Could you check a few things on this model? Use its own coordinates, in mm. Face numbers are marked on the shaded views. A direction names the side the tool comes from. Give positions to 0.01 mm unless a question says otherwise; leave off trailing zeros. Order: outer loops, then holes, each group sorted by start corner. A loop starts at its lowest first (then second) coordinate and runs counter-clockwise, first axis right, second up.
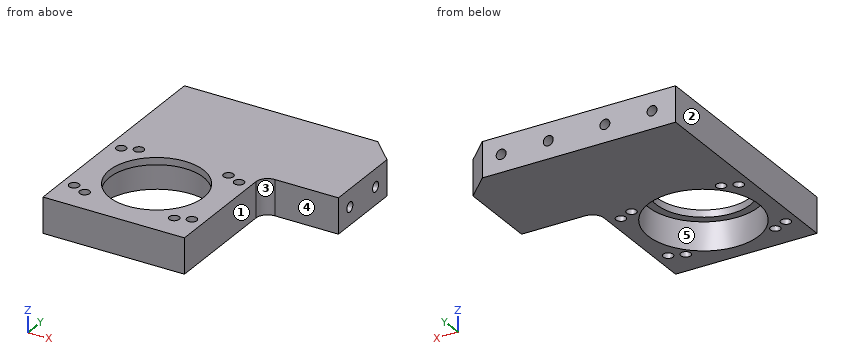
from build123d import *

# Parameters (mm, degrees)
SKETCH_1_W             = 110
SKETCH_1_H             = 100
EXTRUDE_1_DEPTH        = 7.5
SKETCH_10_R            = 23.5
CUT_EXTRUDE_1_DEPTH    = 12
SKETCH_12_R            = 20
CUT_EXTRUDE_2_DEPTH    = 76.292761936
SKETCH_13_W            = 50
SKETCH_13_H            = 55
CUT_EXTRUDE_3_DEPTH    = 76.828754441
FILLET_1_R             = 5
HOLE_WIZARD_M5_1_D     = 4.2
HOLE_WIZARD_M5_2_D     = 4.2
MOVE_FACE_1_BY         = 1
MOVE_FACE_2_BY         = 18
HOLE_WIZARD_M5_3_D     = 4.2
HOLE_WIZARD_M5_3_DEPTH = 12.4
HOLE_WIZARD_M5_3_TIP   = 1.2618073
HOLE_WIZARD_M5_4_D     = 4.2
HOLE_WIZARD_M5_4_DEPTH = 12.4
HOLE_WIZARD_M5_4_TIP   = 1.2618073
CHAMFER_2_SIZE         = 10


with BuildPart() as part:
    # 草图1 → 凸台-拉伸1 (new, symmetric)
    with BuildSketch(Plane.XY):
        Rectangle(SKETCH_1_W, SKETCH_1_H)
    extrude(amount=EXTRUDE_1_DEPTH, both=True)

    # 草图10 → 切除-拉伸1 (cut)
    with BuildSketch(Plane.XY.offset(-7.5)):
        with Locations((-25, -20)):
            Circle(SKETCH_10_R)
    extrude(amount=CUT_EXTRUDE_1_DEPTH, mode=Mode.SUBTRACT)

    # 草图12 → 切除-拉伸2 (cut, through all)
    with BuildSketch(Plane(origin=(0, 0, 4.5), x_dir=(-1, 0, 0), z_dir=(0, 0, -1))):
        with Locations((25, -20)):
            Circle(SKETCH_12_R)
    extrude(amount=-CUT_EXTRUDE_2_DEPTH, mode=Mode.SUBTRACT)

    # 草图13 → 切除-拉伸3 (cut, through all)
    with BuildSketch(Plane.XY.offset(7.5)):
        with Locations((30, -22.5)):
            Rectangle(SKETCH_13_W, SKETCH_13_H)
    extrude(amount=-CUT_EXTRUDE_3_DEPTH, mode=Mode.SUBTRACT)

    # 圆角1
    fillet_1_edges = [part.edges().sort_by_distance(p)[0] for p in [
        (5, 5, 0),
    ]]
    fillet(fillet_1_edges, radius=FILLET_1_R)

    # M5 螺纹孔1 (through all)
    with Locations(Plane(origin=(0, 0, -7.5), x_dir=(-1, 0, 0), z_dir=(0, 0, -1))):
        with Locations((0, -3.5), (0, -36.5), (50, -36.5), (50, -3.5)):
            Hole(HOLE_WIZARD_M5_1_D / 2)

    # M5 螺纹孔2 (through all)
    with Locations(Plane.XY.offset(7.5)):
        with Locations((-44, -1), (-44, -39), (-6, -39), (-6, -1)):
            Hole(HOLE_WIZARD_M5_2_D / 2)

    # Move Face 1: a face moved inward by 1.0
    extrude(part.faces().sort_by_distance((0, 50, 0))[0], amount=MOVE_FACE_1_BY, dir=(0, -1, 0), mode=Mode.SUBTRACT)

    # Move Face 2: a face moved inward by 18.0
    extrude(part.faces().sort_by_distance((55, 27, 0))[0], amount=MOVE_FACE_2_BY, dir=(-1, 0, 0), mode=Mode.SUBTRACT)

    # M5 螺纹孔3
    with Locations(Plane(origin=(0, 49, 0), x_dir=(1, 0, 0), z_dir=(0, 1, 0))):
        with Locations((19, 0), (-1, 0), (-25, 0), (-45, 0)):
            Hole(HOLE_WIZARD_M5_3_D / 2, depth=HOLE_WIZARD_M5_3_DEPTH)
            with Locations((0, 0, -(HOLE_WIZARD_M5_3_DEPTH + HOLE_WIZARD_M5_3_TIP / 2))):  # 118° drill point
                Cone(0, HOLE_WIZARD_M5_3_D / 2, HOLE_WIZARD_M5_3_TIP, mode=Mode.SUBTRACT)

    # M5 螺纹孔4
    with Locations(Plane(origin=(37, 0, 0), x_dir=(0, 0, -1), z_dir=(1, 0, 0))):
        with Locations((0, 13), (0, 31)):
            Hole(HOLE_WIZARD_M5_4_D / 2, depth=HOLE_WIZARD_M5_4_DEPTH)
            with Locations((0, 0, -(HOLE_WIZARD_M5_4_DEPTH + HOLE_WIZARD_M5_4_TIP / 2))):  # 118° drill point
                Cone(0, HOLE_WIZARD_M5_4_D / 2, HOLE_WIZARD_M5_4_TIP, mode=Mode.SUBTRACT)

    # 倒角2
    chamfer_2_edges = [part.edges().sort_by_distance(p)[0] for p in [
        (37, 49, 0),
    ]]
    chamfer(chamfer_2_edges, length=CHAMFER_2_SIZE)


solid = part.part
Item 1: Imagine slicing it at D-D on y = -12.5. List the corners of the cut face in (x, z) for me, then the cut area to 3 significant figures.
Findings:
outline: (-55, -7.5) - (-47.27, -7.5) - (-47.27, 4.5) - (-43.54, 4.5) - (-43.54, 7.5) - (-55, 7.5) - close; (-6.46, 4.5) - (-2.73, 4.5) - (-2.73, -7.5) - (5, -7.5) - (5, 7.5) - (-6.46, 7.5) - close
area: 254 mm2
Item 2: We'd pull the mould along X, two halves only. Please class the marked faces 3, 4 and 5: +X half, -X half, draft (parallel to the pull), parting line (faces both ways), or undercut.
Findings:
face 3: +X half
face 4: draft
face 5: undercut
Item 3: Imagine slicing it at B-B on y = 42.5. List the corners of the cut face in (x, z) for me.
Findings:
outline: (-55, -7.5) - (33.5, -7.5) - (33.5, 7.5) - (-55, 7.5) - close; hole circle Ø4.2 at (-45, 0); hole circle Ø4.2 at (-25, 0); hole circle Ø4.2 at (-1, 0); hole circle Ø4.2 at (19, 0)
Item 4: Imagine slicing it at A-A on z = -4.75. Give the number of separate pieces and of enclosed holes in the cut face, then the cut area to 3 significant figures.
Findings:
separate pieces: 1
enclosed holes: 9
area: 5,460 mm2
Item 5: For pin 1 (14 mm diameter, centred on x = -15.5, y = -18.5, fed in from -Z); pin 2 (3.5 mm diameter, centred on x = -45, z = 0, fed in from +Y); pin 3 (4.5 mm diameter, centred on x = 19, z = 3, fed in from -Y); pin 4 (1.5 mm diameter, centred on y = -14.5, z = 0, fed in from +X), each with a flat end and sliding along its axis, tell me the tip position at first contact or that it passes through.
Findings:
pin 1: passes through
pin 2: stops at y = 36.39
pin 3: stops at y = 5
pin 4: stops at x = 5
Item 6: For the marked faces 1 and 2, which set-ups out of +Z, -Z, +X, -X, +Y, -Y let a thin tool reach every point of the face, with its end or its side?
Findings:
face 1: +Z, -Z, +X, -Y
face 2: +Z, -Z, -X, +Y, -Y
Item 7: Imagine slicing it at C-C on x = -35.5. List the corners of the cut face in (y, z) for me.
Findings:
outline: (-50, -7.5) - (-41.02, -7.5) - (-41.02, 4.5) - (-37.02, 4.5) - (-37.02, 7.5) - (-50, 7.5) - close; (-2.98, 4.5) - (1.02, 4.5) - (1.02, -7.5) - (49, -7.5) - (49, 7.5) - (-2.98, 7.5) - close
Item 8: Please list where these lines run through material, in increasing order: line 1 along Y through (x, z) = (0, -5.5); line 2 along Z through (x, y) = (-25, 39); line 3 along Y through (x, z) = (-49.5, -3.25).
Findings:
line 1: y = -50 to -38.6, -34.4 to -5.6, -1.4 to 49
line 2: z = -7.5 to -2.1, 2.1 to 7.5
line 3: y = -50 to -38.54, -34.46 to -5.54, -1.46 to 49
